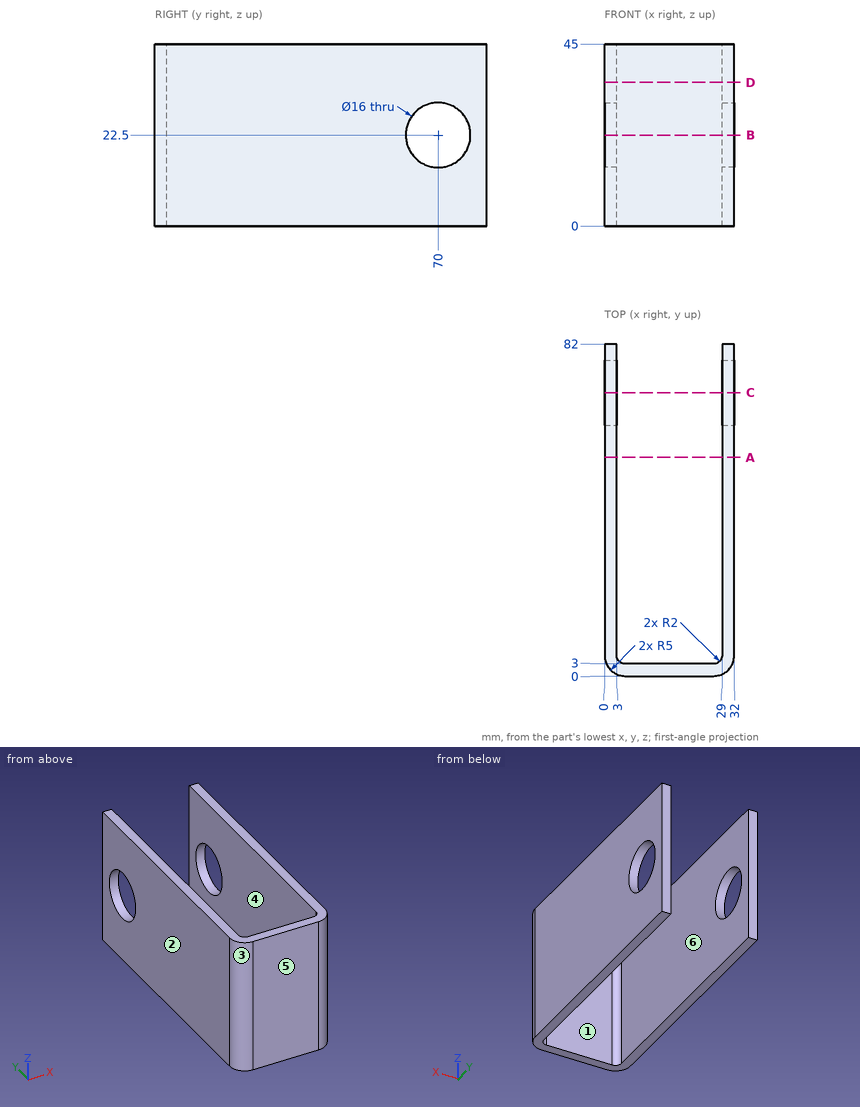
Input: dimensioned drawing with shaded views. Units: mm. Origin: part minimum x, y, z. A direction names the side the tool comes from. Give positions to 0.01 mm unless a question says otherwise; leave off trailing zeros. Write each loop counter-clockwise with the first axis right and the second up, starting at its lowest first coordinate (ties: lowest second). Pieces come first, ordered by that corner, then holes.
1. Material intervals for line 1 along X through (y, z) = (78, 25); line 2 along Y through (x, z) = (30, 22); line 3 along Y through (x, z) = (24.5, 30), sorted ascending.
2. Access query for the marked faces 1 and 2. Directions: +Z, -Z, +X, -X, +Y, -Y. A direction counts if a zero-diameter tool reaches every point of the face in a straight line with its end or side. Return the directions, or none.
3. Section query C-C (y = 70). Return the cut outline in (x, z).
4. Section query A-A (y = 54). Return the cut outline in (x, z), then the cut area to 3 significant figures.
5. Section query B-B (z = 22.5). Return the cut outline in (x, y), then the cut area to 3 significant figures.
6. Section query D-D (z = 35.5). Return the cut outline in (x, y), then the cut area to 3 significant figures.
7. Pull-direction query (X, two-part tool) for the marked faces 3, 4, 5 and 6; classes: +X half, -X half, draft (parallel to the pull), parting line (faces both ways), or undercut.
8. First-contact query: pin 1 (6 mm diameter, centred on x = 17, z = 15, fed in from +Y). Flat tip, straight axial feed; report the tip coordinate or a pass-through.
Output values:
1. line 1: x = 0 to 3, 29 to 32
1. line 2: y = 1 to 62.02, 77.98 to 82
1. line 3: y = 0 to 3
2. face 1: +Z, -Z, +Y
2. face 2: +Z, -Z, -X, +Y, -Y
3. outline: (0, 0) - (3, 0) - (3, 14.5) - (0, 14.5) - close; (0, 30.5) - (3, 30.5) - (3, 45) - (0, 45) - close; (29, 0) - (32, 0) - (32, 14.5) - (29, 14.5) - close; (29, 30.5) - (32, 30.5) - (32, 45) - (29, 45) - close
4. outline: (0, 0) - (3, 0) - (3, 45) - (0, 45) - close; (29, 0) - (32, 0) - (32, 45) - (29, 45) - close
4. area: 270 mm2
5. outline: (0, 5) arc R5 ccw to (5, 0) - (27, 0) arc R5 ccw to (32, 5) - (32, 62) - (29, 62) - (29, 5) arc R2 cw to (27, 3) - (5, 3) arc R2 cw to (3, 5) - (3, 62) - (0, 62) - close; (0, 78) - (3, 78) - (3, 82) - (0, 82) - close; (29, 78) - (32, 78) - (32, 82) - (29, 82) - close
5. area: 465 mm2
6. outline: (0, 5) arc R5 ccw to (5, 0) - (27, 0) arc R5 ccw to (32, 5) - (32, 82) - (29, 82) - (29, 5) arc R2 cw to (27, 3) - (5, 3) arc R2 cw to (3, 5) - (3, 82) - (0, 82) - close
6. area: 561 mm2
7. face 3: -X half
7. face 4: undercut
7. face 5: draft
7. face 6: undercut
8. pin 1: stops at y = 3
